The listing builds one solid part. Answer for the finished solid, in the listing's coordinates (mm). Face numbers are marked on the shaded views. Coordinates: 2 decimals unless noted, no trailing zeros. Order: outer loops, then holes, each group sorted by start corner. A loop starts at its lowest first (then second) coordinate and runs counter-clockwise, first axis right, second up. Notation, with made-up numbers: (-13, 73) -> (5, 73) arc R11 cw to (5, 83) -> close; hole circle Ø2 at (88.25, 20.25). An arc over 180 degrees is marked (long way). Write item = value, one per line.
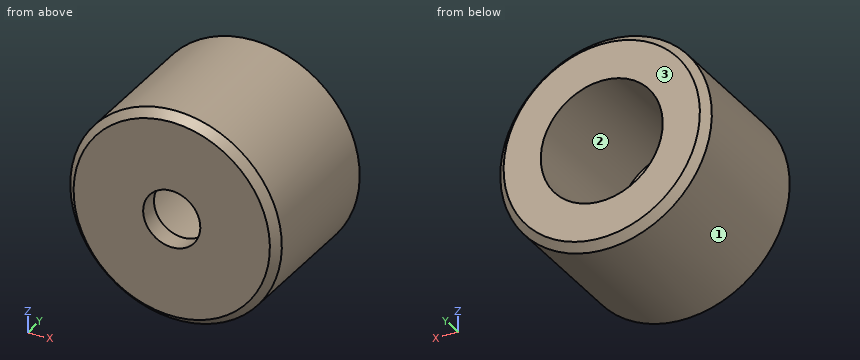
from build123d import *

# Parameters (mm, degrees)
SKETCH_1_R      = 27.75
SKETCH_1_R_2    = 16
EXTRUDE_1_DEPTH = 40
CHAMFER_1_SIZE  = 2
SKETCH_2_R      = 16
SKETCH_2_R_2    = 7.5
EXTRUDE_2_DEPTH = 5


with BuildPart() as part:
    # 草图1 → 凸台-拉伸1 (new body)
    with BuildSketch(Plane(origin=(0, 0, 0), x_dir=(1, 0, 0), z_dir=(0, 1, 0))):
        with Locations(Location((0, 0, 0), (0, 0, 270))):
            Circle(SKETCH_1_R)
        with Locations(Location((0, 0, 0), (0, 0, 270))):
            Circle(SKETCH_1_R_2, mode=Mode.SUBTRACT)
    extrude(amount=EXTRUDE_1_DEPTH)

    # 倒角1
    chamfer_1_edges = [part.edges().sort_by_distance(p)[0] for p in [
        (0, 0, -27.75),
        (0, 40, -27.75),
    ]]
    chamfer(chamfer_1_edges, length=CHAMFER_1_SIZE)

    # 草图2 → 凸台-拉伸2 (add)
    with BuildSketch(Plane.XZ):
        with Locations(Location((0, 0, 0), (0, 0, 270))):
            Circle(SKETCH_2_R)
        with Locations(Location((0, 0, 0), (0, 0, 270))):
            Circle(SKETCH_2_R_2, mode=Mode.SUBTRACT)
    extrude(amount=-EXTRUDE_2_DEPTH)


solid = part.part
Q1. Section A-A, the plane x = 0 is taken. Give the vertices of the cut face in (y, z).
The answers:
outline = (0, -25.75) -> (2, -27.75) -> (38, -27.75) -> (40, -25.75) -> (40, -16) -> (5, -16) -> (5, -7.5) -> (0, -7.5) -> close; (0, 7.5) -> (5, 7.5) -> (5, 16) -> (40, 16) -> (40, 25.75) -> (38, 27.75) -> (2, 27.75) -> (0, 25.75) -> close
Q2. The mould has two halves that part along X. Classify the marked faces 1, 2 and 3: released by +X, released by -X, zero draft, split by the parting line, or undercut.
The answers:
face_1 = split by the parting line
face_2 = undercut
face_3 = zero draft
Q3. Section B-B, the plane z = 0 is taken. Give the vertices of the cut face in (x, y), plus the area to 3 significant figures.
The answers:
outline = (-27.75, 2) -> (-25.75, 0) -> (-7.5, 0) -> (-7.5, 5) -> (-16, 5) -> (-16, 40) -> (-25.75, 40) -> (-27.75, 38) -> close; (7.5, 0) -> (25.75, 0) -> (27.75, 2) -> (27.75, 38) -> (25.75, 40) -> (16, 40) -> (16, 5) -> (7.5, 5) -> close
area = 1,020 mm2
Q4. Section C-C, the plane y = 28.5 is taken. Give the vertices of the cut face in (x, z).
The answers:
outline = circle Ø55.5 at (0, 0); hole circle Ø32 at (0, 0)
Q5. Find the intervals of material crossed by line 1 along X through (y, z) = (28.5, 0); line 2 along Y through (x, z) = (14.5, -5); line 3 along X through (y, z) = (7.5, 14), in increasing order.
The answers:
line_1 = -27.75 to -16, 16 to 27.75
line_2 = 0 to 5
line_3 = -23.96 to -7.75, 7.75 to 23.96
Q6. Each of these flat-tipped pins is pushed along its axis until it touches: pin 1 Ø9 at (x, z) = (0, 0) entering from -Y; pin 2 Ø6 at (x, z) = (-20, 19) entering from +Y; pin 3 Ø10 at (x, y) = (7, 23.5) entering from -Z; pin 4 Ø1.5 at (y, z) = (22.5, 13) entering from +X. Where does it stop, or does it pass through?
The answers:
pin_1 = through
pin_2 = 40
pin_3 = -27.68
pin_4 = 24.9
